Read the model definition and answer for the solid it produces. Units are mm, in the model's axes. A direction names the side the tool comes from. Coordinates: 2 decimals unless noted, no trailing zeros. Write each loop counter-clockwise with the first axis right and the second up, starting at its lowest first coordinate (ties: lowest second). Pieces come first, ordered by that corner, then holes.
1) Each of these flat-tipped pins is pushed along its axis until it touches: pin 1 Ø1.4 at (y, z) = (0, 23) entering from +X; pin 2 Ø4 at (y, z) = (-1, 27) entering from -X; pin 3 Ø1 at (y, z) = (-4.5, 23) entering from +X; pin 4 Ø4 at (y, z) = (1, 29) entering from -X. Where does it stop, or does it pass through?
2) The part is cut by section A-A (z = 17.5). Determine the outline of the cut face in (x, y).
3) The part is cut by section B-B (z = 33). Determine the outline of the cut face in (x, y).
4) Which of the six approach directions +Z, -Z, +X, -X, +Y, -Y give full straight-line access (tool end or side, diameter ignored) to faces 1 (the face through (-4.76, -3.65, 25.03)), 2 (the face through (1.216, 1.115, 30.279)), 3 (the face through (5.5, 0, 24))?
5) Find the intervals of material crossed by line 1 (X direction, y = 0, z = 28.5); line 2 (Y direction, x = 0, z = 28.25), in increasing order.
6) Determine the mould class of faces 4 (the face through (-5.5, 0, 24)), 5 (the face through (2, 0, 35.4)), 6 (the face through (-5.894, 0.259, 7.592)) for opening direction Z: +Z half, -Z half, draft (parallel to the pull), parting line (faces both ways), or undercut.
7) The part is cut by section C-C (z = 10.5). Determine the outline of the cut face in (x, y).
from build123d import *

# Parameters (mm, degrees)
SKETCH1_R               = 5.9
BOSS_EXTRUDE1_DEPTH     = 35.4
M4_TAPPED_HOLE1_D       = 3.3
M4_TAPPED_HOLE1_DEPTH   = 10.1
M4_TAPPED_HOLE1_TIP     = 0.991420021
SKETCH5_R               = 6
SKETCH5_R_2             = 4
BOSS_EXTRUDE2_DEPTH     = 20
CHAMFER1_SIZE           = 1
CUT_EXTRUDE1_DEPTH      = 37.402747149
CUT_EXTRUDE1_DEPTH_BACK = 37.402747149
SKETCH6_W               = 2.026292368
SKETCH6_H               = 10


with BuildPart() as part:
    # Sketch1 → Boss-Extrude1 (new body)
    with BuildSketch(Plane.XY):
        Circle(SKETCH1_R)
    extrude(amount=BOSS_EXTRUDE1_DEPTH)

    # Sketch2 → Revolve1 (revolve)
    with BuildSketch(Plane(origin=(0, 0, 0), x_dir=(1, 0, 0), z_dir=(0, 1, 0))):
        with BuildLine():
            Line((0, 5.9), (0, 0))
            Line((0, 0), (-5.9, 0))
            ThreePointArc((-5.9, 0), (-4.171930009, 4.171930009), (0, 5.9))
        make_face()
    revolve(axis=Axis((0, 0, -5.9), (0, 0, 1)))

    # M4 Tapped Hole1
    with Locations(Plane.XY.offset(35.4)):
        with Locations((0, 0)):
            Hole(M4_TAPPED_HOLE1_D / 2, depth=M4_TAPPED_HOLE1_DEPTH)
            with Locations((0, 0, -(M4_TAPPED_HOLE1_DEPTH + M4_TAPPED_HOLE1_TIP / 2))):  # 118° drill point
                Cone(0, M4_TAPPED_HOLE1_D / 2, M4_TAPPED_HOLE1_TIP, mode=Mode.SUBTRACT)

    # Sketch5 → Boss-Extrude2 (add)
    with BuildSketch(Plane.XY.offset(35.4)):
        Circle(SKETCH5_R)
        Circle(SKETCH5_R_2, mode=Mode.SUBTRACT)
    extrude(amount=-BOSS_EXTRUDE2_DEPTH)

    # Chamfer1
    chamfer1_edges = [part.edges().sort_by_distance(p)[0] for p in [
        (-6, 0, 35.4),
    ]]
    chamfer(chamfer1_edges, length=CHAMFER1_SIZE)

    # Sketch6 → Cut-Extrude1 (cut, two sides: drawn at the far end of the back side and taken through both)
    with BuildSketch(Plane(origin=(0, 0, 0), x_dir=(1, 0, 0), z_dir=(0, 1, 0)).offset(-CUT_EXTRUDE1_DEPTH_BACK)):
        with Locations((-6.513146184, -24.4)):
            Rectangle(SKETCH6_W, SKETCH6_H)
        with Locations((6.513146184, -24.4)):
            Rectangle(SKETCH6_W, SKETCH6_H)
    extrude(amount=CUT_EXTRUDE1_DEPTH + CUT_EXTRUDE1_DEPTH_BACK, mode=Mode.SUBTRACT)


solid = part.part
Reported:
1. pin 1: stops at x = 5.5
1. pin 2: stops at x = -5.5
1. pin 3: stops at x = 4.47
1. pin 4: stops at x = -6
2. outline: circle Ø12 at (0, 0)
3. outline: circle Ø12 at (0, 0); hole circle Ø3.3 at (0, 0)
4. face 1: +Z, -Z
4. face 2: +Z
4. face 3: +X, +Y, -Y
5. line 1: x = -5.5 to -1.65, 1.65 to 5.5
5. line 2: y = -6 to -1.65, 1.65 to 6
6. face 4: undercut
6. face 5: +Z half
6. face 6: draft
7. outline: circle Ø11.8 at (0, 0)
